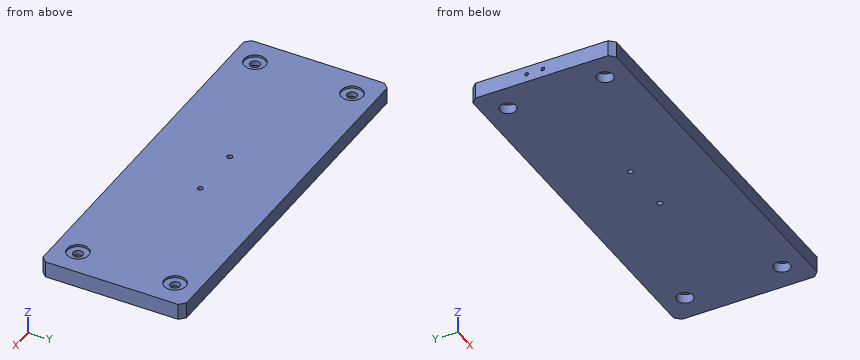
```python
from build123d import *

# Parameters (mm, degrees)
SKETCH1_W                                           = 350
SKETCH1_H                                           = 133
BOSS_EXTRUDE1_DEPTH                                 = 7.5
CBORE_FOR_M8_HEX_SOCKET_HEAD_CAP_SCREW1_D           = 9
CBORE_FOR_M8_HEX_SOCKET_HEAD_CAP_SCREW1_CBORE_D     = 15
CBORE_FOR_M8_HEX_SOCKET_HEAD_CAP_SCREW1_CBORE_DEPTH = 8.6
M6_TAPPED_HOLE1_D                                   = 5
SKETCH6_R                                           = 10
CUT_EXTRUDE1_DEPTH                                  = 2
M4_TAPPED_HOLE1_D                                   = 3.3
M4_TAPPED_HOLE1_DEPTH                               = 10.1
M4_TAPPED_HOLE1_TIP                                 = 0.991420021
CHAMFER1_SIZE                                       = 5


with BuildPart() as part:
    # Sketch1 → Boss-Extrude1 (new, symmetric)
    with BuildSketch(Plane.XY):
        Rectangle(SKETCH1_W, SKETCH1_H)
    extrude(amount=BOSS_EXTRUDE1_DEPTH, both=True)

    # CBORE for M8 Hex Socket Head Cap Screw1 (through all)
    with Locations(Plane(origin=(0, 0, -7.5), x_dir=(-1, 0, 0), z_dir=(0, 0, -1))):
        with Locations((-150, 45), (-150, -45), (150, -45), (150, 45)):
            CounterBoreHole(CBORE_FOR_M8_HEX_SOCKET_HEAD_CAP_SCREW1_D / 2, CBORE_FOR_M8_HEX_SOCKET_HEAD_CAP_SCREW1_CBORE_D / 2, CBORE_FOR_M8_HEX_SOCKET_HEAD_CAP_SCREW1_CBORE_DEPTH)

    # M6 Tapped Hole1 (through all)
    with Locations(Plane.XY.offset(7.5)):
        with Locations((-25, 0), (25, 0)):
            Hole(M6_TAPPED_HOLE1_D / 2)

    # Sketch6 → Cut-Extrude1 (cut)
    with BuildSketch(Plane.XY.offset(7.5)):
        with Locations((-150, 45)):
            Circle(SKETCH6_R)
        with Locations(Location((-150, -45, 0), (0, 0, 180))):
            Circle(SKETCH6_R)
        with Locations((150, -45)):
            Circle(SKETCH6_R)
        with Locations(Location((150, 45, 0), (0, 0, 180))):
            Circle(SKETCH6_R)
    extrude(amount=-CUT_EXTRUDE1_DEPTH, mode=Mode.SUBTRACT)

    # M4 Tapped Hole1
    with Locations(Plane.ZY.offset(175)):
        with Locations((0, 14), (0, -1)):
            Hole(M4_TAPPED_HOLE1_D / 2, depth=M4_TAPPED_HOLE1_DEPTH)
            with Locations((0, 0, -(M4_TAPPED_HOLE1_DEPTH + M4_TAPPED_HOLE1_TIP / 2))):  # 118° drill point
                Cone(0, M4_TAPPED_HOLE1_D / 2, M4_TAPPED_HOLE1_TIP, mode=Mode.SUBTRACT)

    # Chamfer1
    chamfer1_edges = [part.edges().sort_by_distance(p)[0] for p in [
        (175, -66.5, 0),
        (-175, -66.5, 0),
        (-175, 66.5, 0),
        (175, 66.5, 0),
    ]]
    chamfer(chamfer1_edges, length=CHAMFER1_SIZE)


solid = part.part
```
The model under review builds one solid part; all positions refer to its coordinate system, in mm. Give positions to 0.01 mm unless a question says otherwise; leave off trailing zeros. Order: outer loops, then holes, each group sorted by start corner. A loop starts at its lowest first (then second) coordinate and runs counter-clockwise, first axis right, second up. Notation, with made-up numbers: (45.5, 38.25) - (80.5, 38.25) arc R8 ccw to (80.5, 46.25) - close; hole circle Ø5 at (81, -25.5). An arc over 180 degrees is marked (long way). Use CSV: the item, a comma, the result in double quotes. Start each with the question number.
Q1. We need section B-B, the plane y = 45. Write out the cut boundary in (x, z).
Q2. We need section A-A, the plane x = -150. Write out the cut boundary in (y, z).
Q3. Clearance check with flat-ended pins moving along their axes: pin 1 Ø13.5 at (x, y) = (150, -45) entering from -Z; pin 2 Ø12 at (x, y) = (150, 45) entering from +Z; pin 3 Ø8 at (x, y) = (-150, -45) entering from +Z (3 decimals). State where each tip first meets the part, or that it passes through.
Q4. To check wall thickness, follow line 1 along Y through (x, z) = (150, 6.6); line 2 along Y through (x, z) = (150, -5.5); line 3 along X through (y, z) = (-1.5, 5). State the ranges of each line that lie inside material, in increasing order. Write a range as [from, to].
Outcome:
1,outline,"(-175, -7.5) - (-157.5, -7.5) - (-157.5, 1.1) - (-154.5, 1.1) - (-154.5, 5.5) - (-160, 5.5) - (-160, 7.5) - (-175, 7.5) - close; (-145.5, 1.1) - (-142.5, 1.1) - (-142.5, -7.5) - (142.5, -7.5) - (142.5, 1.1) - (145.5, 1.1) - (145.5, 5.5) - (140, 5.5) - (140, 7.5) - (-140, 7.5) - (-140, 5.5) - (-145.5, 5.5) - close; (154.5, 1.1) - (157.5, 1.1) - (157.5, -7.5) - (175, -7.5) - (175, 7.5) - (160, 7.5) - (160, 5.5) - (154.5, 5.5) - close"
2,outline,"(-66.5, -7.5) - (-52.5, -7.5) - (-52.5, 1.1) - (-49.5, 1.1) - (-49.5, 5.5) - (-55, 5.5) - (-55, 7.5) - (-66.5, 7.5) - close; (-40.5, 1.1) - (-37.5, 1.1) - (-37.5, -7.5) - (37.5, -7.5) - (37.5, 1.1) - (40.5, 1.1) - (40.5, 5.5) - (35, 5.5) - (35, 7.5) - (-35, 7.5) - (-35, 5.5) - (-40.5, 5.5) - close; (49.5, 1.1) - (52.5, 1.1) - (52.5, -7.5) - (66.5, -7.5) - (66.5, 7.5) - (55, 7.5) - (55, 5.5) - (49.5, 5.5) - close"
3,pin 1,"stops at z = 1.1"
3,pin 2,"stops at z = 5.5"
3,pin 3,"passes through"
4,line 1,"y = [-66.5, -55], [-35, 35], [55, 66.5]"
4,line 2,"y = [-66.5, -52.5], [-37.5, 37.5], [52.5, 66.5]"
4,line 3,"x = [-175, -27], [-23, 23], [27, 175]"
